For this review, take the finished solid that the model builds, in its own axes (mm). A direction names the side the tool comes from. Round coordinates to 2 decimals unless told otherwise and drop trailing zeros. Order: outer loops, then holes, each group sorted by start corner. A loop starts at its lowest first (then second) coordinate and runs counter-clockwise, first axis right, second up.
```python
from build123d import *

# Parameters (mm, degrees)
CUT_EXTRUDE1_DEPTH = 2.75


with BuildPart() as part:
    # Sketch1 → Revolve1 (revolve)
    with BuildSketch(Plane.XY, mode=Mode.PRIVATE) as revolve1_sk:
        with BuildLine():
            Line((0, 2.5), (-15.8, 2.5))
            ThreePointArc((-15.8, 2.5), (-15.941421356, 2.558578644), (-16, 2.7))
            Line((-16, 2.7), (-16, 4.75))
            ThreePointArc((-16, 4.75), (-17.581194586, 3.877015605), (-18.75, 2.5))
            Line((-18.75, 2.5), (-18.75, 0))
            Line((-18.75, 0), (0, 0))
            Line((0, 0), (0, 2.5))
        make_face()
    revolve(revolve1_sk.sketch.rotate(Axis((-18.75, 0, 0), (1, 0, 0)), 90), axis=Axis((-18.75, 0, 0), (1, 0, 0)))

    # Sketch2 → Cut-Extrude1 (cut)
    with BuildSketch(Plane.ZY.offset(18.75)):
        Polygon((0, 1.732050808), (-1.5, 0.866025404), (-1.5, -0.866025404), (0, -1.732050808), (1.5, -0.866025404), (1.5, 0.866025404), align=None)
    extrude(amount=-CUT_EXTRUDE1_DEPTH, mode=Mode.SUBTRACT)

    # Sketch6 → Revolve2 (revolve)
    with BuildSketch(Plane.XY):
        Polygon((-17.19, 1.732050808), (-16, 0), (-15.56, 0), (-15.56, 1.732050808), align=None)
    revolve(axis=Axis((-18.75, 0, 0), (1, 0, 0)))

    # Sketch7 → Cut-Revolve5 (revolve, cut)
    with BuildSketch(Plane.XY):
        Polygon((-18.75, 1.732050808), (-18.31, 0), (-18.75, 0), align=None)
    revolve(axis=Axis((-18.75, 0, 0), (1, 0, 0)), mode=Mode.SUBTRACT)

    # Sketch4 → Cut-Revolve1 (revolve, cut)
    with BuildSketch(Plane.XY, mode=Mode.PRIVATE) as cut_revolve1_sk:
        Polygon((-0.4, 2.5), (0, 1.807179677), (0.4, 2.5), align=None)
    revolve(cut_revolve1_sk.sketch.rotate(Axis((-0.4, 0, 0), (1, 0, 0)), 90), axis=Axis((-0.4, 0, 0), (1, 0, 0)), mode=Mode.SUBTRACT)


solid = part.part
```
Q1. Take a section at A-A, the plane x = -9.75. State the section outline as (y, z) points.
Q2. Tool access review of faces 4 (the face through (-18, 0, -1.5)), 5 (the face through (-16, 2.04, -2.04)), 6 (the face through (0, 0, 0)): name each direction out of +Z, -Z, +X, -X, +Y, -Y from which nothing blocks a thin tool from reaching the whole face with its end or side.
Q3. Clearance check with flat-ended pins moving along their axes: pin 1 (1.5 mm diameter, centred on x = -14, y = -0.5, fed in from -Z); pin 2 (5 mm diameter, centred on x = -5.5, z = -3.5, fed in from -Y); pin 3 (1 mm diameter, centred on y = -3.5, z = -1.5, fed in from +X). State where each tip first meets the part, or that it passes through.
Q4. Take a section at B-B, the plane y = -3.5. State the section outline as (x, z) points, plus the area to 3 significant figures.
Q5. Wall thickness on line 1 (Y direction, x = -10.5, z = 2); line 2 (Z direction, x = -11, y = 2.25): over which ranges is each line inside the solid? List them lowest first.
Q6. Mouldability with a two-part tool opening along Z and no side actions: class faces 1 (the face through (-8.2, -0.1, -2.5)), 2 (the face through (-18.75, -1, 2)), 3 (the face through (-17.902, -1.305, 0.74)) as +Z half, -Z half, draft (parallel to the pull), parting line (faces both ways), or undercut.
Working result:
1. outline: circle Ø5 at (0, 0)
2. face 4: -X
2. face 5: +X
2. face 6: +Z, -Z, +X, +Y, -Y
3. pin 1: stops at z = -2.5
3. pin 2: stops at y = -2.29
3. pin 3: stops at x = -16
4. outline: (-16, -3.21) - (-16, 3.21) arc R3.58 ccw to start
4. area: 9.16 mm2
5. line 1: y = -1.5 to 1.5
5. line 2: z = -1.09 to 1.09
6. face 1: parting line
6. face 2: draft
6. face 3: undercut
